```python
from build123d import *

# Parameters (mm, degrees)
BOSS_EXTRUDE1_DEPTH = 1


with BuildPart() as part:
    # Sketch1 → Boss-Extrude1 (new, symmetric)
    with BuildSketch(Plane.XY):
        with BuildLine():
            Line((-76.2, 508), (76.2, 508))
            ThreePointArc((76.2, 508), (183.963073453, 463.363073453), (228.6, 355.6))
            Line((228.6, 355.6), (228.6, 0))
            Line((228.6, 0), (-228.6, 0))
            Line((-228.6, 0), (-228.6, 355.6))
            ThreePointArc((-228.6, 355.6), (-183.963073453, 463.363073453), (-76.2, 508))
        make_face()
        with BuildLine():
            Line((-101.6, 309.88), (101.6, 309.88))
            ThreePointArc((101.6, 309.88), (137.521024484, 295.001024484), (152.4, 259.08))
            Line((152.4, 259.08), (152.4, 208.28))
            ThreePointArc((152.4, 208.28), (137.521024484, 172.358975516), (101.6, 157.48))
            Line((101.6, 157.48), (-101.6, 157.48))
            ThreePointArc((-101.6, 157.48), (-137.521024484, 172.358975516), (-152.4, 208.28))
            Line((-152.4, 208.28), (-152.4, 259.08))
            ThreePointArc((-152.4, 259.08), (-137.521024484, 295.001024484), (-101.6, 309.88))
        make_face(mode=Mode.SUBTRACT)
    extrude(amount=BOSS_EXTRUDE1_DEPTH, both=True)


solid = part.part
```
For this review, take the finished solid that the model builds, in its own axes (mm). A direction names the side the tool comes from. Coordinates: 2 decimals unless noted, no trailing zeros. Write each loop counter-clockwise with the first axis right and the second up, starting at its lowest first coordinate (ties: lowest second). Pieces come first, ordered by that corner, then holes. Notation, with made-up numbers: (57, 78) - (89, 78) arc R26 ccw to (89, 115) - close; hole circle Ø8 at (-17, 22). An arc over 180 degrees is marked (long way). Answer in a Markdown table with one row per item. Add a question column.
Q1. Draft analysis for pull direction X (two halves, no side actions). For faces 1 (the cylindrical face through (182.772, 464.541, 0.014)), 2 (the flat face through (3, 314, -1)), 3 (the cylindrical face through (137.124, 295.394, 0.014)), state which applies: +X half, -X half, draft (parallel to the pull), parting line (faces both ways), or undercut.
Q2. For probe 1 along Y at (x, z) = (24.5, 0.9); probe 2 along X at (y, z) = (256, 0.45); probe 3 along Y at (x, z) = (-99, 0.8), list the stretches that pass through material, from the lowest coordinate up.
Q3. We need section B-B, the plane z = -0.3. State the section outline as (x, y) points.
Q4. Tool access review of faces 4 (the flat face through (3, 314, 1)), 5 (the cylindrical face through (137.914, 172.756, 0.014)): name each direction out of +Z, -Z, +X, -X, +Y, -Y from which nothing blocks a thin tool from reaching the whole face with its end or side.
Q5. We need section C-C, the plane y = 276. State the section outline as (x, z) points.
Q6. We need section A-A, the plane x = -62.5. State the section outline as (y, z) points.
Q7. We need section D-D, the plane x = -189. State the section outline as (y, z) points.
Answer list:
| question | item | result |
|---|---|---|
| 1 | face 1 | +X half |
| 1 | face 2 | draft |
| 1 | face 3 | undercut |
| 2 | probe 1 | y = 0 to 157.48, 309.88 to 508 |
| 2 | probe 2 | x = -228.6 to -152.4, 152.4 to 228.6 |
| 2 | probe 3 | y = 0 to 157.48, 309.88 to 506.28 |
| 3 | outline | (-228.6, 0) - (228.6, 0) - (228.6, 355.6) arc R152.4 ccw to (76.2, 508) - (-76.2, 508) arc R152.4 ccw to (-228.6, 355.6) - close; hole (-152.4, 208.28) arc R50.8 ccw to (-101.6, 157.48) - (101.6, 157.48) arc R50.8 ccw to (152.4, 208.28) - (152.4, 259.08) arc R50.8 ccw to (101.6, 309.88) - (-101.6, 309.88) arc R50.8 ccw to (-152.4, 259.08) - close |
| 4 | face 4 | +Z, +X, -X, +Y, -Y |
| 4 | face 5 | +Z, -Z |
| 5 | outline | (-228.6, -1) - (-149.5, -1) - (-149.5, 1) - (-228.6, 1) - close; (149.5, -1) - (228.6, -1) - (228.6, 1) - (149.5, 1) - close |
| 6 | outline | (0, -1) - (157.48, -1) - (157.48, 1) - (0, 1) - close; (309.88, -1) - (508, -1) - (508, 1) - (309.88, 1) - close |
| 7 | outline | (0, -1) - (458.08, -1) - (458.08, 1) - (0, 1) - close |
